For this review, use the dimensioned drawing (mm, ordinates from the lowest corner) and the shaded views. Round coordinates to 2 decimals unless told otherwise and drop trailing zeros. Write each loop counter-clockwise with the first axis right and the second up, starting at its lowest first coordinate (ties: lowest second). Pieces come first, ordered by that corner, then holes. Notation, with made-up numbers: M 5,88.5 L 13,88.5 A25 cw 13,115.5 Z; hole C -14,59 d1. An arc over 180 degrees is marked long. Use CSV: the item, a comma, the result in double quotes.
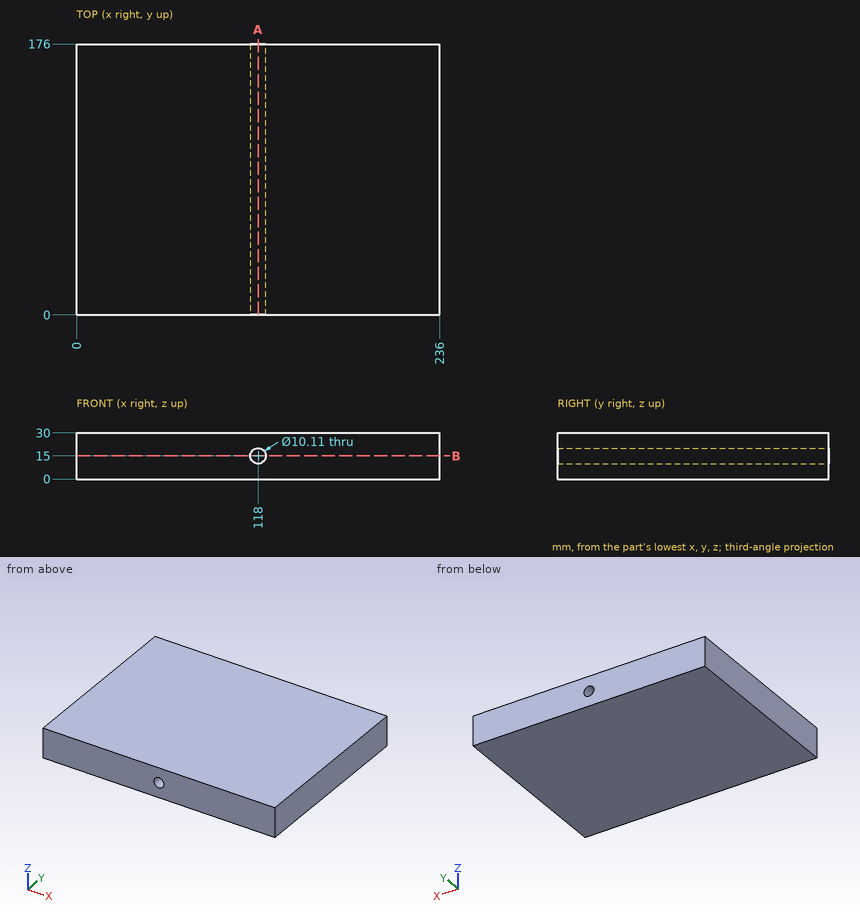
1) Add section B-B on z = 15. Write out the cut boundary in (x, y) (3 decimals), then the cut area to 3 significant figures.
Answers:
outline,"M 0,0 L 112.945,0 L 112.945,176 L 0,176 Z; M 123.055,0 L 236,0 L 236,176 L 123.055,176 Z"
area,"39,800 mm²"
2) Add section A-A on x = 118. Write out the cut boundary in (y, z) (3 decimals), then the cut area to 3 significant figures.
Answers:
outline,"M 0,0 L 176,0 L 176,9.945 L 0,9.945 Z; M 0,20.055 L 176,20.055 L 176,30 L 0,30 Z"
area,"3,500 mm²"
3) Wall thickness on line 1 along Z through (x, y) = (118, 99.5) (3 decimals); line 2 along X through (y, z) = (62.5, 13); line 3 along X through (y, z) = (153, 16): over which ranges is each line inside the solid? List them lowest first. Write a range as [from, to].
Answers:
line 1,"[0, 9.945], [20.055, 30]"
line 2,"[0, 113.36], [122.64, 236]"
line 3,"[0, 113.04], [122.96, 236]"
